Could you check a few things on this model? Use its own coordinates, in mm. A direction names the side the tool comes from. Round coordinates to 2 decimals unless told otherwise and drop trailing zeros. Order: outer loops, then holes, each group sorted by start corner. A loop starts at its lowest first (then second) coordinate and runs counter-clockwise, first axis right, second up. Notation, with made-up numbers: M -24,-1.75 L -11,-1.75 A9 cw -11,8.25 Z; hole C 15,87.25 d2. An arc over 180 degrees is marked long. Write each question's results on one line, items separated by ' | '. Start each with the question number.
1. For faces 4 (the flat face through (-92, -5, -10)), 5 (the flat face through (-92.9, -38.3, -20)), which set-ups out of +Z, -Z, +X, -X, +Y, -Y let a thin tool reach every point of the face, with its end or its side?
2. I'm going to push a flat-ended pin straight in: pin 1 (10 mm diameter, centred on x = -99, y = -26.5, fed in from -Z). Where does the tip first touch, or does it pass through?
3. Suppose I cut it at C-C on y = -11. Write out the boundary of the cut face in (x, z).
4. Suppose I cut it at B-B on x = -106. Write out the boundary of the cut face in (y, z).
5. Please list where these lines run through material, in increasing order: L1, parallel to X at y = -22, z = -3.5; L2, parallel to Y at x = -105, z = -9.75; L3, parallel to Z at x = -86, y = -15.
6. Suppose I cut it at A-A on z = -7.25. Write out the boundary of the cut face in (x, y).
7. We'd pull the mould along Y, two halves only. Please class faces 1 (the flat face through (-92, -4, -10)), 2 (the flat face through (-109, -22, -10)), 3 (the flat face through (-92, -21, -1)): released by +Y, released by -Y, zero draft, split by the parting line, or undercut.
from build123d import *

# Parameters (mm, degrees)
SKETCH1_W           = 35
SKETCH1_H           = 35
BOSS_EXTRUDE1_DEPTH = 20
SHELL1_T            = -1


with BuildPart() as part:
    # Sketch1 → Boss-Extrude1 (new body)
    with BuildSketch(Plane.XY):
        with Locations((-91.5, -21.5)):
            Rectangle(SKETCH1_W, SKETCH1_H)
    extrude(amount=-BOSS_EXTRUDE1_DEPTH)

    # Shell1
    shell1_openings = [part.faces().sort_by_distance(p)[0] for p in [
        (-91.5, -21.5, -20),
    ]]
    offset(amount=SHELL1_T, openings=shell1_openings, kind=Kind.INTERSECTION)


solid = part.part
Filled sheet:
1) face 4: -Z | face 5: -Z, +X, -X, +Y, -Y
2) pin 1: stops at z = -1
3) outline: M -109,-20 L -108,-20 L -108,-1 L -75,-1 L -75,-20 L -74,-20 L -74,0 L -109,0 Z
4) outline: M -39,-20 L -38,-20 L -38,-1 L -5,-1 L -5,-20 L -4,-20 L -4,0 L -39,0 Z
5) L1: x = -109 to -108, -75 to -74 | L2: y = -39 to -38, -5 to -4 | L3: z = -1 to 0
6) outline: M -109,-39 L -74,-39 L -74,-4 L -109,-4 Z; hole M -108,-38 L -75,-38 L -75,-5 L -108,-5 Z
7) face 1: released by +Y | face 2: zero draft | face 3: undercut
